The model under review builds one solid part; all positions refer to its coordinate system, in mm. A direction names the side the tool comes from. Coordinates: 2 decimals unless noted, no trailing zeros. Loops run counter-clockwise (first coordinate to the right, second up) from the corner with the lowest first, then second, coordinate; pieces in that order, holes last. Notation, with made-up numbers: M 85.25,21.25 L 134.25,21.25 A7 cw 134.25,30.25 Z; hole C 29.5,44 d10. An arc over 180 degrees is marked long. One line per item, written item: value.
```python
from build123d import *

# Parameters (mm, degrees)
SKETCH2_OUTSIDE_W   = 40.868
SKETCH2_OUTSIDE_H   = 40.868
SKETCH2_OUTSIDE_W_2 = 26.310212334
SKETCH2_OUTSIDE_H_2 = 15
CUT_EXTRUDE1_DEPTH  = 30
SKETCH3_R           = 2.5
CUT_EXTRUDE2_DEPTH  = 5
CUT_EXTRUDE3_START  = -5
SKETCH5_R           = 2.5
CUT_EXTRUDE3_DEPTH  = 5


with BuildPart() as part:
    # Sketch1 → Revolve1 (revolve)
    with BuildSketch(Plane.XY, mode=Mode.PRIVATE) as revolve1_sk:
        Polygon((-1.5, -45.854266644), (-1.5, 44.145733356), (-4.5, 44.145733356), (-10, 24.145733356), (-10, -13.854266644), (-8, -13.854266644), (-8, -23.854266644), (-10, -23.854266644), (-10, -28.854266644), (-9, -28.854266644), (-9, -34.854266644), (-8.2, -34.854266644), (-8.2, -36.854266644), (-9, -36.854266644), (-9, -42.854266644), (-8.77234172, -45.854266644), align=None)
    revolve(revolve1_sk.sketch.rotate(Axis((0, 0, 0), (0, 1, 0)), 270), axis=Axis((0, 0, 0), (0, 1, 0)))

    # Sketch2 outside → Cut-Extrude1 (cut)
    with BuildSketch(Plane(origin=(0, -45.854266644, 0), x_dir=(-1, 0, 0), z_dir=(0, -1, 0))):
        Rectangle(SKETCH2_OUTSIDE_W, SKETCH2_OUTSIDE_H)
        Rectangle(SKETCH2_OUTSIDE_W_2, SKETCH2_OUTSIDE_H_2, mode=Mode.SUBTRACT)
    extrude(amount=-CUT_EXTRUDE1_DEPTH, mode=Mode.SUBTRACT)

    # Sketch3 → Cut-Extrude2 (cut)
    with BuildSketch(Plane.XY.offset(7.5)):
        with Locations((0, -35.854266644)):
            Circle(SKETCH3_R)
    extrude(amount=-CUT_EXTRUDE2_DEPTH, mode=Mode.SUBTRACT)

    # Sketch5 → Cut-Extrude3 (cut)
    with BuildSketch(Plane(origin=(0, 0, -7.5), x_dir=(-1, 0, 0), z_dir=(0, 0, -1)).offset(CUT_EXTRUDE3_START)):
        with Locations(Location((0, -35.854266644, 0), (0, 0, 180))):
            Circle(SKETCH5_R)
    extrude(amount=CUT_EXTRUDE3_DEPTH, mode=Mode.SUBTRACT)


solid = part.part
```
(1) Add section D-D on y = 29.5. State the section outline as (x, z) points, then the cut area to 3 significant figures.
Checks:
outline: C 0,0 d17.06; hole C 0,0 d3
area: 221 mm^2
(2) Add section C-C on y = 5. State the section outline as (x, z) points.
Checks:
outline: C 0,0 d20; hole C 0,0 d3
(3) Draft analysis for pull direction X (two halves, no side actions). For faces 1 (the face through (0, -36, -2.5)), 2 (the face through (-9.2, -28.854, 0)), 3 (the face through (10, -26, 0)), state which applies: pulls with the +X half, pulls with the -X half, needs draft (parallel to the pull), parting line crosses it, or undercut.
Checks:
face 1: undercut
face 2: needs draft
face 3: pulls with the +X half
(4) To check wall thickness, follow L1, parallel to Z at x = 2.5, y = -27; L2, parallel to X at y = 18, z = -0.25; L3, parallel to X at y = -23.5, z = -0.5. State the ranges of each line that lie inside material, in increasing order. Write a range as [from, to].
Checks:
L1: [-7.5, 7.5]
L2: [-10, -1.48], [1.48, 10]
L3: [-7.98, -1.41], [1.41, 7.98]
(5) Add section B-B on x = 0. State the section outline as (y, z) points.
Checks:
outline: M -45.85,-7.5 L -38.35,-7.5 L -38.35,-2.5 L -33.35,-2.5 L -33.35,-7.5 L -15.85,-7.5 L -15.85,-8 L -13.85,-8 L -13.85,-10 L 24.15,-10 L 44.15,-4.5 L 44.15,-1.5 L -45.85,-1.5 Z; M -45.85,1.5 L 44.15,1.5 L 44.15,4.5 L 24.15,10 L -13.85,10 L -13.85,8 L -15.85,8 L -15.85,7.5 L -33.35,7.5 L -33.35,2.5 L -38.35,2.5 L -38.35,7.5 L -45.85,7.5 Z
(6) Insertion check: pin 1 Ø1.5 at (y, z) = (6, -2.5) entering from -X; pin 2 Ø12 at (x, y) = (-6, -25) entering from +Z; pin 3 Ø8 at (x, y) = (-4.5, -14.5) entering from +Z; pin 4 Ø1.7 at (x, z) = (5, 0.5) entering from +Y. Each pin has a flat end and moves straight along its axis. Give the tip position at first contact, or say it passes through.
Checks:
pin 1: x = -9.85
pin 2: z = 7.5
pin 3: z = 9.98
pin 4: y = 44.15
(7) Tool access review of faces 4 (the face through (0, -31, 7.5)), 5 (the face through (7.81, -18.92, 1.73)), 6 (the face through (9, -40, 0)), 7 (the face through (8.2, -35.9, 0.1)), 8 (the face through (-9, -40, 0)): name each direction out of +Z, -Z, +X, -X, +Y, -Y from which nothing blocks a thin tool from reaching the whole face with its end or side.
Checks:
face 4: +Z, +X, -X, -Y
face 5: none
face 6: +X, -Y
face 7: +X
face 8: -X, -Y
